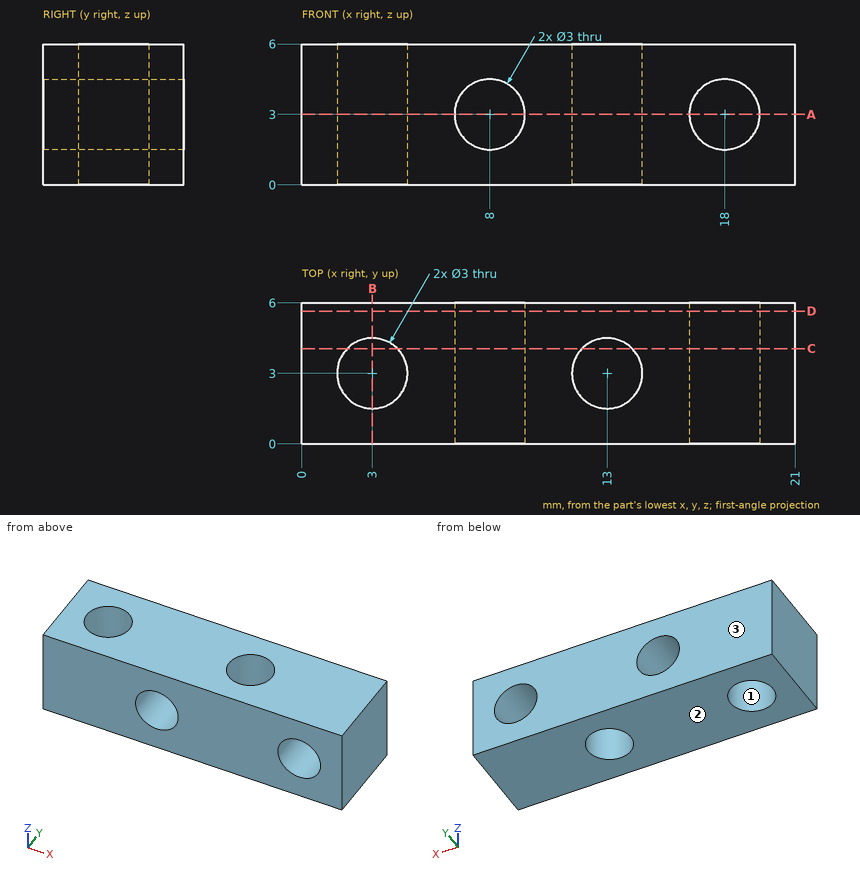
Source: three-view drawing plus pictorial views. Frame: mm from the lowest corner of the part. Give positions to 0.01 mm unless a question says otherwise; leave off trailing zeros. Loops run counter-clockwise (first coordinate to the right, second up) from the corner with the lowest first, then second, coordinate; pieces in that order, holes last. Notation, with made-up numbers: (70, -31.75) -> (94, -31.75) arc R20 cw to (94, -6.75) -> close; hole circle Ø7 at (39.25, 3.5). An arc over 180 degrees is marked (long way). Put each result on its own line as item: value. Start each with the question number.
1) Cut plane A-A (z = 3). Return loops of the section in (x, y), then the cut area to 3 significant figures.
2) Cut plane C-C (y = 4.05). Return loops of the section in (x, z), then the cut area to 3 significant figures.
3) Draft query along Y for the marked faces 1, 2 and 3. Return one class per face: released by +Y, released by -Y, zero draft, split by the parting line, or undercut.
4) Cut plane D-D (y = 5.65). Return loops of the section in (x, z), then the cut area to 3 significant figures.
5) Material intervals for probe 1 along X at (y, z) = (2.95, 5.55); probe 2 along X at (y, z) = (1.25, 3); probe 3 along Z at (x, y) = (8, 1.95), sorted ascending.
6) Cut plane B-B (x = 3). Return loops of the section in (y, z).
7) Contact query for a flat-ended pin moving along its axis: P1, Ø2.5, axis at x = 13, y = 3, coming from the +Z side. Output: stop coordinate, or through.
Results are:
1. outline: (0, 0) -> (6.5, 0) -> (6.5, 6) -> (0, 6) -> close; (9.5, 0) -> (16.5, 0) -> (16.5, 6) -> (9.5, 6) -> close; (19.5, 0) -> (21, 0) -> (21, 6) -> (19.5, 6) -> close; hole circle Ø3 at (3, 3); hole circle Ø3 at (13, 3)
1. area: 75.9 mm2
2. outline: (0, 0) -> (1.93, 0) -> (1.93, 6) -> (0, 6) -> close; (4.07, 0) -> (11.93, 0) -> (11.93, 6) -> (4.07, 6) -> close; (14.07, 0) -> (21, 0) -> (21, 6) -> (14.07, 6) -> close; hole circle Ø3 at (8, 3); hole circle Ø3 at (18, 3)
2. area: 86.2 mm2
3. face 1: undercut
3. face 2: zero draft
3. face 3: released by +Y
4. outline: (0, 0) -> (21, 0) -> (21, 6) -> (0, 6) -> close; hole circle Ø3 at (8, 3); hole circle Ø3 at (18, 3)
4. area: 112 mm2
5. probe 1: x = 0 to 1.5, 4.5 to 11.5, 14.5 to 21
5. probe 2: x = 0 to 6.5, 9.5 to 16.5, 19.5 to 21
5. probe 3: z = 0 to 1.5, 4.5 to 6
6. outline: (0, 0) -> (1.5, 0) -> (1.5, 6) -> (0, 6) -> close; (4.5, 0) -> (6, 0) -> (6, 6) -> (4.5, 6) -> close
7. P1: passes through
